Check sheet for the modelled part. Datum: model origin and axes. Units: mm. A direction names the side the tool comes from. Round coordinates to 2 decimals unless told otherwise and drop trailing zeros. Order: outer loops, then holes, each group sorted by start corner. A loop starts at its lowest first (then second) coordinate and runs counter-clockwise, first axis right, second up.
(1) Thickness scan on probe 1 along X at (y, z) = (19, 1); probe 2 along Y at (x, z) = (18.5, -11.5); probe 3 along X at (y, z) = (25.5, 16.5). Record the ranges inside material, lowest first.
(2) Tool access check on faces 4 (the flat face through (20, 14, 0)), 5 (the flat face through (-13, 13, -19)), 6 (the flat face through (49, 7, -7)). Record the directions out of +Z, -Z, +X, -X, +Y, -Y that give a thin tool (end or side, any length) a straight path to the whole face; none if there is none.
(3) Sectioned sample at A-A, the plane x = 48.5. Enter the section's corners in (y, z), and give its area (3 significant figures).
(4) Sectioned sample at D-D, the plane x = 37. Enter the section's corners in (y, z), and give its area (3 significant figures).
(5) Sectioned sample at C-C, the plane z = 0. Enter the section's corners in (x, y), and give its area (3 significant figures).
(6) Sectioned sample at B-B, the plane y = 18.5. Enter the section's corners in (x, z).
(7) Depth check by flat-ended pin: pin 1 (3 mm diameter, centred on x = 24.5, z = 14.5, fed in from -Y); pin 2 (2.5 mm diameter, centred on y = 17.5, z = 17, fed in from -X); pin 3 (6 mm diameter, centred on x = 51, z = 9.5, fed in from +Y); pin 4 (2.5 mm diameter, centred on x = -18, y = 10, fed in from +Z). Enter the tip coordinate at first touch or a pass-through.
(8) Mould release check, pull along Z, two halves, no side actions. Record for faces 1 (the flat face through (-11.13, 27.23, -13.33)), 2 (the cylindrical face through (31, 7, 0)), 3 (the flat face through (-4, 20, 0)): released by +Z, released by -Z, zero draft, split by the parting line, or undercut.
```python
from build123d import *

# Parameters (mm, degrees)
SLOTTED_BASE_PLATE_DEPTH = 14
UPRIGHT_BLOCK_DEPTH      = 9
TOP_STEP_BOSS_DEPTH      = 9


with BuildPart() as part:
    # Base Plate Profile Sketch → Slotted Base Plate (new body)
    with BuildSketch(Plane(origin=(0, 0, 0), x_dir=(1, 0, 0), z_dir=(0, 1, 0))):
        Polygon((-22, -15), (-13, -15), (-13, -23), (22, -23), (22, 23), (-13, 23), (-13, 15), (-22, 15), align=None)
        with BuildLine():
            ThreePointArc((38, 7), (31, 0), (38, -7))
            Line((38, -7), (60, -7))
            Line((60, -7), (60, -18))
            Line((60, -18), (22, -23))
            Line((22, -23), (22, 23))
            Line((22, 23), (60, 18))
            Line((60, 18), (60, 7))
            Line((60, 7), (38, 7))
        make_face()
    extrude(amount=SLOTTED_BASE_PLATE_DEPTH)

    # Upright Block Sketch → Upright Block (add)
    with BuildSketch(Plane.ZY.offset(22)):
        Polygon((7, 30), (-7, 30), (-15, 26.5), (-15, 0), (15, 0), (15, 26.5), align=None)
    extrude(amount=-UPRIGHT_BLOCK_DEPTH)

    # Top Step Sketch → Top Step Boss (add)
    with BuildSketch(Plane.ZY.offset(13)):
        Polygon((-7, 30), (7, 30), (23, 23), (23, 0), (-23, 0), (-23, 23), align=None)
    extrude(amount=-TOP_STEP_BOSS_DEPTH)


solid = part.part
```
Derived:
1. probe 1: x = -22 to -4
1. probe 2: y = 0 to 14
1. probe 3: x = -13 to -4
2. face 4: +Z, -Z, +X, +Y
2. face 5: -Z, -X, +Y, -Y
2. face 6: +X, +Y, -Y
3. outline: (0, -19.51) - (14, -19.51) - (14, -7) - (0, -7) - close; (0, 7) - (14, 7) - (14, 19.51) - (0, 19.51) - close
3. area: 350 mm2
4. outline: (0, -21.03) - (14, -21.03) - (14, -6.93) - (0, -6.93) - close; (0, 6.93) - (14, 6.93) - (14, 21.03) - (0, 21.03) - close
4. area: 395 mm2
5. outline: (-22, 0) - (31, 0) - (31, 14) - (-4, 14) - (-4, 30) - (-22, 30) - close
5. area: 1,030 mm2
6. outline: (-22, -15) - (-13, -15) - (-13, -23) - (-4, -23) - (-4, 23) - (-13, 23) - (-13, 15) - (-22, 15) - close
7. pin 1: stops at y = 0
7. pin 2: stops at x = -13
7. pin 3: stops at y = 14
7. pin 4: stops at z = 15
8. face 1: released by -Z
8. face 2: undercut
8. face 3: zero draft
